```python
from build123d import *

# Parameters (mm, degrees)
BOSS_EXTRUDE1_DEPTH = 35
CHAMFER1_SIZE       = 1


with BuildPart() as part:
    # Sketch1 → Boss-Extrude1 (new body)
    with BuildSketch(Plane(origin=(0, 0, 0), x_dir=(1, 0, 0), z_dir=(0, 1, 0))):
        with BuildLine():
            Line((-2, 7.5), (2, 7.5))
            ThreePointArc((2, 7.5), (9.5, 0), (2, -7.5))
            Line((2, -7.5), (-2, -7.5))
            ThreePointArc((-2, -7.5), (-9.5, 0), (-2, 7.5))
        make_face()
    extrude(amount=BOSS_EXTRUDE1_DEPTH)

    # Chamfer1
    chamfer1_edges = [part.edges().sort_by_distance(p)[0] for p in [
        (9.5, 35, 0),
        (0, 35, -7.5),
        (-9.5, 35, 0),
        (0, 0, -7.5),
        (9.5, 0, 0),
        (0, 0, 7.5),
        (-9.5, 0, 0),
        (0, 35, 7.5),
    ]]
    chamfer(chamfer1_edges, length=CHAMFER1_SIZE)


solid = part.part
```
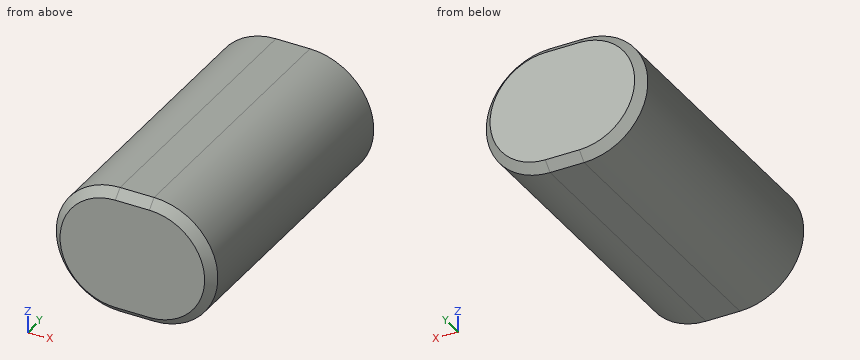
Geometry check sheet. Reference: the model listing, model coordinates, mm. Round coordinates to 2 decimals unless told otherwise and drop trailing zeros. Loops run counter-clockwise (first coordinate to the right, second up) from the corner with the lowest first, then second, coordinate; pieces in that order, holes last. Notation, with made-up numbers: (-5, 35) - (53, 35) arc R36 cw to (53, 70) - close; hole circle Ø9 at (-34, -14.75). An arc over 180 degrees is marked (long way). Write item = value, one per line. Start each with the question number.
1. Section check A-A on y = 29.5. Enter the section's corners in (x, z), then the cut area to 3 significant figures.
2. Thickness scan on line 1 (X direction, y = 14, z = -6.25); line 2 (X direction, y = 22, z = -3.25); line 3 (Z direction, x = 7.75, y = 16). Record the ranges inside material, lowest first.
3. Depth check by flat-ended pin: pin 1 (10 mm diameter, centred on x = -7.5, y = 27, fed in from -Z); pin 2 (2 mm diameter, centred on x = -3.5, y = 3.5, fed in from +Z); pin 3 (2 mm diameter, centred on x = 5, y = 13.5, fed in from -Z). Enter the tip coordinate at first touch or a pass-through.
Working result:
q1.outline = (-2, -7.5) - (2, -7.5) arc R7.5 ccw to (2, 7.5) - (-2, 7.5) arc R7.5 ccw to start
q1.area = 237 mm^2
q2.line_1 = -6.15 to 6.15
q2.line_2 = -8.76 to 8.76
q2.line_3 = -4.82 to 4.82
q3.pin_1 = -7.48
q3.pin_2 = 7.48
q3.pin_3 = -7.23
